Work out the finished part from the listing and answer in its coordinate system (mm). Face numbers are marked on the shaded views. A direction names the side the tool comes from. Round coordinates to 2 decimals unless told otherwise and drop trailing zeros. Order: outer loops, then holes, each group sorted by start corner. A loop starts at its lowest first (then second) coordinate and runs counter-clockwise, first axis right, second up. Notation, with made-up numbers: (30.5, -0.5) -> (61.5, -0.5) arc R31 cw to (61.5, 38.5) -> close; hole circle Ø7 at (47.5, -38). An arc over 180 degrees is marked (long way). Use a Markdown table: item, result. Add a question column.
Item 1: A cutting plane is placed at B-B, the plane z = 26. Determine the outline of the cut face in (x, y).
Item 2: A cutting plane is placed at D-D, the plane z = 2. Determine the outline of the cut face in (x, y).
Item 3: A tool of negligible diameter and unlimited length cuts with its end or side. For the marked faces 1, 2 and 3, from which of +Z, -Z, +X, -X, +Y, -Y can it reach the whole face along a straight path? Write none if from no direction.
Item 4: Find the intervals of material crossed by L1, parallel to X at y = 47, z = 12; L2, parallel to Y at x = -33, z = 15, in increasing order. Write a range as [from, to].
Item 5: A cutting plane is placed at A-A, the plane z = 7.5. Determine the outline of the cut face in (x, y), plus the area to 3 significant figures.
Item 6: Flat-ended cylindrical pins translate along their axes: P1, Ø13.5, axis at y = 9.5, z = 19, coming from the -X side; P2, Ø5, axis at x = -27.5, z = 5.5, coming from the -Y side; P3, Ø3, axis at y = 27, z = 10.5, coming from the +X side. Find the tip coordinate at first contact, or state that the pin passes through.
Item 7: A cutting plane is placed at C-C, the plane x = -13.5. Determine the outline of the cut face in (y, z), plus the area to 3 significant figures.
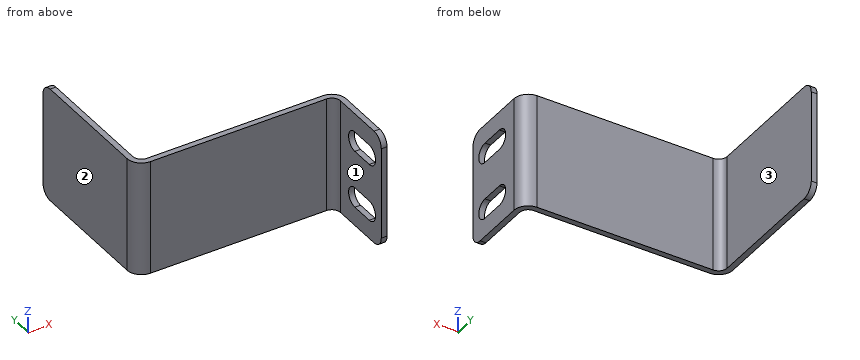
from build123d import *

# Parameters (mm, degrees)
EXTRUDE_1_DEPTH     = 30
FILLET_1_R          = 3
CUT_EXTRUDE_1_DEPTH = 10


with BuildPart() as part:
    # 草图1 → 拉伸-薄壁1 (new body)
    with BuildSketch(Plane.XY):
        with BuildLine():
            Line((0.75, 0), (0.75, 17))
            ThreePointArc((0.75, 17), (-0.348349571, 19.651650429), (-3, 20.75))
            Line((-3, 20.75), (-49, 20.75))
            ThreePointArc((-49, 20.75), (-50.590990258, 21.409009742), (-51.25, 23))
            Line((-51.25, 23), (-51.25, 58))
            Line((-51.25, 58), (-52.75, 58))
            Line((-52.75, 58), (-52.75, 23))
            ThreePointArc((-52.75, 23), (-51.651650429, 20.348349571), (-49, 19.25))
            Line((-49, 19.25), (-3, 19.25))
            ThreePointArc((-3, 19.25), (-1.409009742, 18.590990258), (-0.75, 17))
            Line((-0.75, 17), (-0.75, 0))
            Line((-0.75, 0), (0.75, 0))
        make_face()
    extrude(amount=EXTRUDE_1_DEPTH)

    # 圆角1
    fillet_1_edges = [part.edges().sort_by_distance(p)[0] for p in [
        (0, 0, 0),
        (-52, 58, 0),
        (0, 0, 30),
        (-52, 58, 30),
    ]]
    fillet(fillet_1_edges, radius=FILLET_1_R)

    # 草图2 → 切除-拉伸1 (cut)
    with BuildSketch(Plane.ZY.offset(0.75)):
        with BuildLine():
            Line((10.1, 11), (10.1, 5))
            ThreePointArc((10.1, 5), (7.5, 2.4), (4.9, 5))
            Line((4.9, 5), (4.9, 11))
            ThreePointArc((4.9, 11), (7.5, 13.6), (10.1, 11))
        make_face()
        with BuildLine():
            Line((25.1, 11), (25.1, 5))
            ThreePointArc((25.1, 5), (22.5, 2.4), (19.9, 5))
            Line((19.9, 5), (19.9, 11))
            ThreePointArc((19.9, 11), (22.5, 13.6), (25.1, 11))
        make_face()
    extrude(amount=-CUT_EXTRUDE_1_DEPTH, mode=Mode.SUBTRACT)


solid = part.part
Reported:
| question | item | result |
|---|---|---|
| 1 | outline | (-52.75, 23) arc R3.75 ccw to (-49, 19.25) -> (-3, 19.25) arc R2.25 cw to (-0.75, 17) -> (-0.75, 0) -> (0.75, 0) -> (0.75, 17) arc R3.75 ccw to (-3, 20.75) -> (-49, 20.75) arc R2.25 cw to (-51.25, 23) -> (-51.25, 58) -> (-52.75, 58) -> close |
| 2 | outline | (-52.75, 23) arc R3.75 ccw to (-49, 19.25) -> (-3, 19.25) arc R2.25 cw to (-0.75, 17) -> (-0.75, 0.17) -> (0.75, 0.17) -> (0.75, 17) arc R3.75 ccw to (-3, 20.75) -> (-49, 20.75) arc R2.25 cw to (-51.25, 23) -> (-51.25, 57.83) -> (-52.75, 57.83) -> close |
| 3 | face 1 | +Z, -Z, -X, -Y |
| 3 | face 2 | +Z, -Z, -X, +Y, -Y |
| 3 | face 3 | +Z, -Z, +X, +Y |
| 4 | L1 | [-52.75, -51.25] |
| 4 | L2 | [19.25, 20.75] |
| 5 | outline | (-52.75, 23) arc R3.75 ccw to (-49, 19.25) -> (-3, 19.25) arc R2.25 cw to (-0.75, 17) -> (-0.75, 13.6) -> (0.75, 13.6) -> (0.75, 17) arc R3.75 ccw to (-3, 20.75) -> (-49, 20.75) arc R2.25 cw to (-51.25, 23) -> (-51.25, 58) -> (-52.75, 58) -> close; (-0.75, 0) -> (0.75, 0) -> (0.75, 2.4) -> (-0.75, 2.4) -> close |
| 5 | area | 144 mm² |
| 6 | P1 | x = -0.75 |
| 6 | P2 | y = 19.25 |
| 6 | P3 | x = -51.25 |
| 7 | outline | (19.25, 0) -> (20.75, 0) -> (20.75, 30) -> (19.25, 30) -> close |
| 7 | area | 45.0 mm² |
